```python
from build123d import *

# Parameters (mm, degrees)
BOSS_EXTRUDE1_DEPTH        = 80
SKETCH2_R                  = 2.75
CUT_EXTRUDE1_DEPTH         = 10
SKETCH3_W                  = 314
SKETCH3_H                  = 25
CUT_EXTRUDE2_DEPTH         = 10
SKETCH4_W                  = 140
SKETCH4_H                  = 50
BOSS_EXTRUDE2_DEPTH        = 3
SKETCH5_W                  = 24.712329927
SKETCH5_H                  = 27.5
CUT_EXTRUDE3_DEPTH         = 15
CHAMFER1_SIZE              = 5
CHAMFER2_SIZE              = 8
CUT_EXTRUDE4_DEPTH         = 112
SKETCH9_R                  = 1
CUT_EXTRUDE5_DEPTH         = 10
M4_TAPPED_HOLE1_AT_2_COUNT = 2
M4_TAPPED_HOLE1_AT_2_PITCH = 24
LPATTERN1_COUNT            = 3
LPATTERN1_PITCH            = 60
SKETCH11_R                 = 2.25
CUT_EXTRUDE6_DEPTH         = 10
LPATTERN2_COUNT            = 3
LPATTERN2_PITCH            = 25
CHAMFER3_SIZE              = 5
CHAMFER4_SIZE              = 5
FILLET1_R                  = 5


with BuildPart() as part:
    # Sketch1 → Boss-Extrude1 (new body)
    with BuildSketch(Plane(origin=(0, 0, 0), x_dir=(1, 0, 0), z_dir=(0, 1, 0))):
        Polygon((0, 0), (18, 0), (18, 3), (3, 3), (3, 160), (0, 160), align=None)
    extrude(amount=BOSS_EXTRUDE1_DEPTH)

    # Sketch2 → Cut-Extrude1 (cut)
    with BuildSketch(Plane.XY):
        with Locations((10, 40)):
            Circle(SKETCH2_R)
    extrude(amount=-CUT_EXTRUDE1_DEPTH, mode=Mode.SUBTRACT)

    # Sketch3 → Cut-Extrude2 (cut)
    with BuildSketch(Plane.ZY):
        with Locations((-160, 40)):
            Rectangle(SKETCH3_W, SKETCH3_H)
    extrude(amount=-CUT_EXTRUDE2_DEPTH, mode=Mode.SUBTRACT)

    # Sketch4 → Boss-Extrude2 (add)
    with BuildSketch(Plane.ZY):
        with Locations((70, 40)):
            Rectangle(SKETCH4_W, SKETCH4_H)
    extrude(amount=-BOSS_EXTRUDE2_DEPTH)

    # Sketch5 → Cut-Extrude3 (cut)
    with BuildSketch(Plane(origin=(18, 0, 0), x_dir=(0, 0, -1), z_dir=(1, 0, 0))):
        with Locations((-2.356164964, 13.75)):
            Rectangle(SKETCH5_W, SKETCH5_H)
        with Locations((-2.356164964, 66.25)):
            Rectangle(SKETCH5_W, SKETCH5_H)
    extrude(amount=-CUT_EXTRUDE3_DEPTH, mode=Mode.SUBTRACT)

    # Chamfer1
    chamfer1_edges = [part.edges().sort_by_distance(p)[0] for p in [
        (18, 27.5, -1.5),
        (18, 52.5, -1.5),
    ]]
    chamfer(chamfer1_edges, length=CHAMFER1_SIZE)

    # Chamfer2
    chamfer2_edges = [part.edges().sort_by_distance(p)[0] for p in [
        (1.5, 0, 0),
        (1.5, 80, 0),
    ]]
    chamfer(chamfer2_edges, length=CHAMFER2_SIZE)

    # Sketch8 → Cut-Extrude4 (cut)
    with BuildSketch(Plane(origin=(0, 0, -3), x_dir=(-1, 0, 0), z_dir=(0, 0, -1))):
        with BuildLine():
            Line((-26, 43.1), (-10, 43.1))
            ThreePointArc((-10, 43.1), (-6.9, 40), (-10, 36.9))
            Line((-10, 36.9), (-26, 36.9))
            ThreePointArc((-26, 36.9), (-29.1, 40), (-26, 43.1))
        make_face()
    extrude(amount=-CUT_EXTRUDE4_DEPTH, mode=Mode.SUBTRACT)

    # Sketch9 → Cut-Extrude5 (cut)
    with BuildSketch(Plane.ZY):
        with Locations((133, 52)):
            Circle(SKETCH9_R)
        with Locations((133, 28)):
            Circle(SKETCH9_R)
    extrude(amount=-CUT_EXTRUDE5_DEPTH, mode=Mode.SUBTRACT)

    # Sketch10 → M4 Tapped Hole1 (revolve, cut)
    with BuildSketch(Plane(origin=(0, 52, 133), x_dir=(0, 0, 1), z_dir=(0, 1, 0))):
        Polygon((0, 0), (0, 11.091420021), (1.65, 10.1), (1.65, 0), align=None)
    m4_tapped_hole1 = revolve(axis=Axis((-6.35, 52, 133), (1, 0, 0)), mode=Mode.SUBTRACT)

    # M4 Tapped Hole1 at 2: M4 Tapped Hole1 ×2
    with Locations(*[(0, -i * M4_TAPPED_HOLE1_AT_2_PITCH, 0) for i in range(1, M4_TAPPED_HOLE1_AT_2_COUNT)]):
        add(m4_tapped_hole1, mode=Mode.SUBTRACT)

    # LPattern1: M4 Tapped Hole1 ×3
    with Locations(*[(0, 0, -i * LPATTERN1_PITCH) for i in range(1, LPATTERN1_COUNT)]):
        add(m4_tapped_hole1, mode=Mode.SUBTRACT)

    # LPattern1 copy 1 sketch → LPattern1 copy 1 (revolve, cut)
    with BuildSketch(Plane(origin=(0, 28, 73), x_dir=(0, 0, 1), z_dir=(0, 1, 0))):
        Polygon((0, 0), (0, 11.091420021), (1.65, 10.1), (1.65, 0), align=None)
    revolve(axis=Axis((-6.35, 28, 73), (1, 0, 0)), mode=Mode.SUBTRACT)

    # LPattern1 copy 2 sketch → LPattern1 copy 2 (revolve, cut)
    with BuildSketch(Plane(origin=(0, 28, 13), x_dir=(0, 0, 1), z_dir=(0, 1, 0))):
        Polygon((0, 0), (0, 11.091420021), (1.65, 10.1), (1.65, 0), align=None)
    revolve(axis=Axis((-6.35, 28, 13), (1, 0, 0)), mode=Mode.SUBTRACT)

    # Sketch11 → Cut-Extrude6 (cut)
    with BuildSketch(Plane.ZY):
        with Locations((-155, 70)):
            Circle(SKETCH11_R)
        with Locations((-155, 10)):
            Circle(SKETCH11_R)
    cut_extrude6 = extrude(amount=-CUT_EXTRUDE6_DEPTH, mode=Mode.SUBTRACT)

    # LPattern2: Cut-Extrude6 ×3
    with Locations(*[(0, 0, i * LPATTERN2_PITCH) for i in range(1, LPATTERN2_COUNT)]):
        add(cut_extrude6, mode=Mode.SUBTRACT)

    # Chamfer3
    chamfer3_edges = [part.edges().sort_by_distance(p)[0] for p in [
        (1.5, 52.5, -160),
        (1.5, 27.5, -160),
    ]]
    chamfer(chamfer3_edges, length=CHAMFER3_SIZE)

    # Chamfer4
    chamfer4_edges = [part.edges().sort_by_distance(p)[0] for p in [
        (1.5, 15, 140),
        (1.5, 65, 140),
    ]]
    chamfer(chamfer4_edges, length=CHAMFER4_SIZE)

    # Fillet1
    fillet1_edges = [part.edges().sort_by_distance(p)[0] for p in [
        (1.5, 15, 0),
        (1.5, 65, 0),
    ]]
    fillet(fillet1_edges, radius=FILLET1_R)


solid = part.part
```
Model file for the job. Use its own axes, mm. A direction names the side the tool comes from. Round coordinates to 2 decimals unless told otherwise and drop trailing zeros. Order: outer loops, then holes, each group sorted by start corner. A loop starts at its lowest first (then second) coordinate and runs counter-clockwise, first axis right, second up. Notation, with made-up numbers: (72.5, 54) -> (114.5, 54) arc R5 ccw to (114.5, 62) -> close; hole circle Ø4 at (23.25, 78.5). An arc over 180 degrees is marked (long way). Use one line per item in the form item = value.
Item 1: Flat gauge pins, fed straight in: pin 1 Ø1.5 at (x, z) = (1, 57) entering from -Y; pin 2 Ø2 at (x, y) = (1, 71) entering from +Z; pin 3 Ø3.5 at (x, z) = (12.5, -1) entering from -Y. Where does each tip first touch, or does it go through?
Returned:
pin_1 = 15
pin_2 = 0
pin_3 = 27.5
Item 2: Cut at C-C, the plane z = 88. Write the cut outline in (x, y).
Returned:
outline = (0, 15) -> (3, 15) -> (3, 65) -> (0, 65) -> close
Item 3: Tool access for faces 5 (the face through (0, 57, -12)), 6 (the face through (1.5, 55, -157.5)), 7 (the face through (8.7, 37, 0)): list every direction of +Z, -Z, +X, -X, +Y, -Y with a clear straight run to the whole face (end or side of a thin tool).
Returned:
face_5 = +Z, -Z, -X, +Y, -Y
face_6 = -Z, +X, -X
face_7 = +Z, +X, +Y, -Y
Item 4: Pull direction Y, two halves, no side cores. Call faces 1 (the face through (1.5, 25, -157.5)), 2 (the face through (1, 76, -4)), 3 (the face through (5, 40, -3)), 4 (the face through (1, 4, -4)): released by +Y, released by -Y, zero draft, split by the parting line, or undercut.
Returned:
face_1 = undercut
face_2 = released by +Y
face_3 = undercut
face_4 = released by -Y
Item 5: Drill centre lines: line 1 (Y direction, x = 1.25, z = -130); line 2 (Y direction, x = 1.15, z = 13); line 3 (Y direction, x = 1.25, z = -69.5). Where is each one in solid material? Low to high.
Returned:
line_1 = 0 to 7.75, 12.25 to 27.5, 52.5 to 67.75, 72.25 to 80
line_2 = 15 to 26.35, 29.65 to 50.35, 53.65 to 65
line_3 = 0 to 27.5, 52.5 to 80
Item 6: Cut at B-B, the plane y = 40. Write the cut outline in (x, z).
Returned:
outline = (0, -3) -> (6.9, -3) -> (6.9, 0) -> (3, 0) -> (3, 140) -> (0, 140) -> close
Item 7: Cut at A-A, the plane z = -42.5. Write the cut outline in (x, y), and give its area (3 significant figures).
Returned:
outline = (0, 0) -> (3, 0) -> (3, 27.5) -> (0, 27.5) -> close; (0, 52.5) -> (3, 52.5) -> (3, 80) -> (0, 80) -> close
area = 165 mm^2
